Input: part model. Units: mm. Frame: model coordinates. Face numbers are marked on the shaded views. Round coordinates to 2 decimals unless told otherwise and drop trailing zeros. Write each loop counter-clockwise with the first axis right and the second up, starting at its lowest first coordinate (ties: lowest second). Pieces come first, ordered by that corner, then holes. Notation, with made-up numbers: (-21, 64) -> (31, 64) arc R18 ccw to (31, 81) -> close; hole circle Ø3 at (82.25, 89.5). An arc over 180 degrees is marked (long way). Write item = value, one per line.
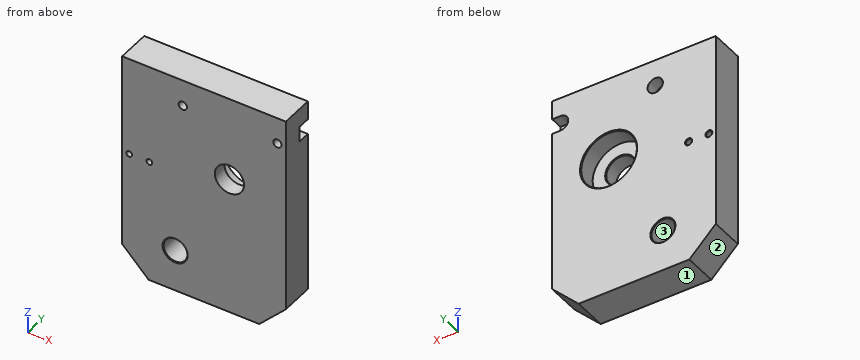
```python
from build123d import *

# Parameters (mm, degrees)
BOSS_EXTRUDE1_DEPTH         = 24
SKETCH_2_2_R                = 8.5
SKETCH_2_2_R_2              = 20
SKETCH_2_2_R_3              = 3
CUT_EXTRUDE1_DEPTH          = 13
SKETCH_2_2_2_R              = 8.5
SKETCH_2_2_2_R_2            = 3
CUT_EXTRUDE2_DEPTH          = 103.311411876
SKETCH3_R                   = 10.5
CUT_EXTRUDE3_DEPTH          = 101.302666964
M5_TAPPED_HOLE1_D           = 4.2
M5_TAPPED_HOLE1_CSINK_D     = 5.05
M5_TAPPED_HOLE1_CSINK_ANGLE = 90
CHAMFER1_SIZE               = 0.5
CUT_EXTRUDE4_START          = -24
SKETCH6_R                   = 5.5
SKETCH6_R_2                 = 3
SKETCH6_W                   = 5.693229178
SKETCH6_H                   = 11
CUT_EXTRUDE4_DEPTH          = 9
CHAMFER2_SIZE               = 0.5


with BuildPart() as part:
    # Sketch1 → Boss-Extrude1 (new body)
    with BuildSketch(Plane(origin=(0, 0, 0), x_dir=(1, 0, 0), z_dir=(0, 1, 0))):
        Polygon((-58.75, 61.25), (-39.75, 80.25), (39.75, 80.25), (58.75, 61.25), (58.75, -80.25), (-58.75, -80.25), align=None)
    extrude(amount=BOSS_EXTRUDE1_DEPTH)

    # Sketch 2_2 → Cut-Extrude1 (cut)
    with BuildSketch(Plane(origin=(0, 24, 0), x_dir=(1, 0, 0), z_dir=(0, 1, 0))):
        with Locations(Location((-20.75, 50.25, 0), (0, 0, 270))):
            Circle(SKETCH_2_2_R)
        with Locations(Location((18.25, -19.75, 0), (0, 0, 270))):
            Circle(SKETCH_2_2_R_2)
        with Locations(Location((52.75, -61.25, 0), (0, 0, 270))):
            Circle(SKETCH_2_2_R_3)
        with Locations(Location((-15.25, -61.25, 0), (0, 0, 270))):
            Circle(SKETCH_2_2_R_3)
    extrude(amount=-CUT_EXTRUDE1_DEPTH, mode=Mode.SUBTRACT)

    # Sketch 2_2 2 → Cut-Extrude2 (cut, through all)
    with BuildSketch(Plane(origin=(0, 24, 0), x_dir=(1, 0, 0), z_dir=(0, 1, 0))):
        with Locations(Location((-20.75, 50.25, 0), (0, 0, 270))):
            Circle(SKETCH_2_2_2_R)
        with Locations(Location((52.75, -61.25, 0), (0, 0, 270))):
            Circle(SKETCH_2_2_2_R_2)
        with Locations(Location((-15.25, -61.25, 0), (0, 0, 270))):
            Circle(SKETCH_2_2_2_R_2)
    extrude(amount=-CUT_EXTRUDE2_DEPTH, mode=Mode.SUBTRACT)

    # Sketch3 → Cut-Extrude3 (cut, through all)
    with BuildSketch(Plane(origin=(0, 11, 0), x_dir=(1, 0, 0), z_dir=(0, 1, 0))):
        with Locations(Location((18.25, -19.75, 0), (0, 0, 270))):
            Circle(SKETCH3_R)
    extrude(amount=-CUT_EXTRUDE3_DEPTH, mode=Mode.SUBTRACT)

    # M5 Tapped Hole1 (through all)
    with Locations(Plane(origin=(0, 24, 0), x_dir=(1, 0, 0), z_dir=(0, 1, 0))):
        with Locations((-39.25, -8.75), (-53.75, -8.75)):
            CounterSinkHole(M5_TAPPED_HOLE1_D / 2, M5_TAPPED_HOLE1_CSINK_D / 2, counter_sink_angle=M5_TAPPED_HOLE1_CSINK_ANGLE)

    # Chamfer1
    chamfer1_edges = [part.edges().sort_by_distance(p)[0] for p in [
        (-20.75, 24, -58.75),
        (18.25, 24, -0.25),
        (-20.75, 0, -58.75),
        (18.25, 11, 9.25),
    ]]
    chamfer(chamfer1_edges, length=CHAMFER1_SIZE)

    # Sketch6 → Cut-Extrude4 (cut)
    # profile 1 of 7: a face of its own
    with BuildSketch(Plane.XZ.offset(CUT_EXTRUDE4_START)):
        with Locations(Location((-15.25, 61.25, 0), (0, 0, 90))):
            Circle(SKETCH6_R)
        with Locations(Location((-15.25, 61.25, 0), (0, 0, 90))):
            Circle(SKETCH6_R_2, mode=Mode.SUBTRACT)
    # profile 2 of 7: a face of its own
    with BuildSketch(Plane.XZ.offset(CUT_EXTRUDE4_START)):
        with BuildLine():
            ThreePointArc((58.25, 61.25), (56.639087297, 65.139087297), (52.75, 66.75))
            ThreePointArc((52.75, 66.75), (52.40269227, 66.73902335), (52.056770822, 66.706137215))
            Line((52.056770822, 66.706137215), (52.056770822, 64.168806829))
            ThreePointArc((52.056770822, 64.168806829), (54.610149519, 63.603687271), (55.75, 61.25))
            ThreePointArc((55.75, 61.25), (54.610149519, 58.896312729), (52.056770822, 58.331193171))
            Line((52.056770822, 58.331193171), (52.056770822, 55.793862785))
            ThreePointArc((52.056770822, 55.793862785), (52.40269227, 55.76097665), (52.75, 55.75))
            ThreePointArc((52.75, 55.75), (56.639087297, 57.360912703), (58.25, 61.25))
        make_face()
    # profile 3 of 7: a face of its own
    with BuildSketch(Plane.XZ.offset(CUT_EXTRUDE4_START)):
        with BuildLine():
            Line((52.056770822, 64.168806829), (52.056770822, 66.706137215))
            ThreePointArc((52.056770822, 66.706137215), (47.25, 61.25), (52.056770822, 55.793862785))
            Line((52.056770822, 55.793862785), (52.056770822, 58.331193171))
            ThreePointArc((52.056770822, 58.331193171), (49.75, 61.25), (52.056770822, 64.168806829))
        make_face()
    # profile 4 of 7: a face of its own
    with BuildSketch(Plane.XZ.offset(CUT_EXTRUDE4_START)):
        with Locations((61.596614589, 61.25)):
            Rectangle(SKETCH6_W, SKETCH6_H)
    # profile 5 of 7: a face of its own
    with BuildSketch(Plane.XZ.offset(CUT_EXTRUDE4_START)):
        with BuildLine():
            ThreePointArc((58.25, 61.25), (56.639087297, 65.139087297), (52.75, 66.75))
            ThreePointArc((52.75, 66.75), (52.40269227, 66.73902335), (52.056770822, 66.706137215))
            Line((52.056770822, 66.706137215), (52.056770822, 64.168806829))
            ThreePointArc((52.056770822, 64.168806829), (54.610149519, 63.603687271), (55.75, 61.25))
            ThreePointArc((55.75, 61.25), (54.610149519, 58.896312729), (52.056770822, 58.331193171))
            Line((52.056770822, 58.331193171), (52.056770822, 55.793862785))
            ThreePointArc((52.056770822, 55.793862785), (52.40269227, 55.76097665), (52.75, 55.75))
            ThreePointArc((52.75, 55.75), (56.639087297, 57.360912703), (58.25, 61.25))
        make_face()
    # profile 6 of 7: a face of its own
    with BuildSketch(Plane.XZ.offset(CUT_EXTRUDE4_START)):
        with BuildLine():
            Line((52.056770822, 64.168806829), (52.056770822, 66.706137215))
            ThreePointArc((52.056770822, 66.706137215), (47.25, 61.25), (52.056770822, 55.793862785))
            Line((52.056770822, 55.793862785), (52.056770822, 58.331193171))
            ThreePointArc((52.056770822, 58.331193171), (49.75, 61.25), (52.056770822, 64.168806829))
        make_face()
    # profile 7 of 7: a face of its own
    with BuildSketch(Plane.XZ.offset(CUT_EXTRUDE4_START)):
        with BuildLine():
            Line((58.75, 66.75), (52.75, 66.75))
            ThreePointArc((52.75, 66.75), (56.639087297, 65.139087297), (58.25, 61.25))
            ThreePointArc((58.25, 61.25), (56.639087297, 57.360912703), (52.75, 55.75))
            Line((52.75, 55.75), (58.75, 55.75))
            Line((58.75, 55.75), (58.75, 66.75))
        make_face()
    extrude(amount=CUT_EXTRUDE4_DEPTH, mode=Mode.SUBTRACT)

    # Chamfer2
    chamfer2_edges = [part.edges().sort_by_distance(p)[0] for p in [
        (52.75, 15, 58.25),
    ]]
    chamfer(chamfer2_edges, length=CHAMFER2_SIZE)


solid = part.part
```
1) Cut plane D-D (y = 17.75). Return the cut outline in (x, z).
Solutions:
outline = (-58.75, -61.25) -> (-39.75, -80.25) -> (39.75, -80.25) -> (58.75, -61.25) -> (58.75, 55.75) -> (52.75, 55.75) arc R5.5 cw to (52.75, 66.75) -> (58.75, 66.75) -> (58.75, 80.25) -> (-58.75, 80.25) -> close; hole circle Ø4.2 at (-53.75, 8.75); hole circle Ø4.2 at (-39.25, 8.75); hole circle Ø17 at (-20.75, -50.25); hole circle Ø11 at (-15.25, 61.25); hole circle Ø40 at (18.25, 19.75)
2) Cut plane C-C (y = 6.75). Return the cut outline in (x, z), and give its area (3 significant figures).
Solutions:
outline = (-58.75, -61.25) -> (-39.75, -80.25) -> (39.75, -80.25) -> (58.75, -61.25) -> (58.75, 80.25) -> (-58.75, 80.25) -> close; hole circle Ø4.2 at (-53.75, 8.75); hole circle Ø4.2 at (-39.25, 8.75); hole circle Ø17 at (-20.75, -50.25); hole circle Ø6 at (-15.25, 61.25); hole circle Ø21 at (18.25, 19.75); hole circle Ø6 at (52.75, 61.25)
area = 17,800 mm^2
3) Cut plane B-B (z = 19.75). Return the cut outline in (x, y).
Solutions:
outline = (-58.75, 0) -> (7.75, 0) -> (7.75, 10.5) -> (7.25, 11) -> (-1.75, 11) -> (-1.75, 23.5) -> (-2.25, 24) -> (-58.75, 24) -> close; (28.75, 0) -> (58.75, 0) -> (58.75, 24) -> (38.75, 24) -> (38.25, 23.5) -> (38.25, 11) -> (29.25, 11) -> (28.75, 10.5) -> close
4) Line query: L1, parallel to X at y = 11.5, z = 61.25; L2, parallel to X at y = 19.5, z = 19.75; L3, parallel to X at y = 13, z = -50.5. Output: solid intervals per line, ascending. Write a range as from..to.
Solutions:
L1 = -58.75..-18.25, -12.25..49.75, 55.75..58.75
L2 = -58.75..-1.75, 38.25..58.75
L3 = -58.75..-29.25, -12.25..58.75
5) First-contact query: P1, Ø3, axis at x = 55, y = 18, coming from the -Z side. Flat tip, straight axial feed; report the tip coordinate or a pass-through.
Solutions:
P1 = -66.5
6) Draft query along X for the marked faces 1, 2 and 3. Return one class per face: +X half, -X half, draft (parallel to the pull), parting line (faces both ways), or undercut.
Solutions:
face_1 = draft
face_2 = -X half
face_3 = undercut
7) Cut plane A-A (x = 18.25). Return the cut outline in (y, z), and give its area (3 significant figures).
Solutions:
outline = (0, -80.25) -> (24, -80.25) -> (24, -0.75) -> (23.5, -0.25) -> (11, -0.25) -> (11, 8.75) -> (10.5, 9.25) -> (0, 9.25) -> close; (0, 30.25) -> (10.5, 30.25) -> (11, 30.75) -> (11, 39.75) -> (23.5, 39.75) -> (24, 40.25) -> (24, 80.25) -> (0, 80.25) -> close
area = 3,100 mm^2
